Part model, mm, in its own coordinate system. A direction names the side the tool comes from. Give positions to 0.01 mm unless a question says otherwise; leave off trailing zeros. Order: outer loops, then holes, each group sorted by start corner. A loop starts at its lowest first (then second) coordinate and runs counter-clockwise, first axis right, second up. Notation, with made-up numbers: M 67.5,41 L 110.5,41 A15 ccw 110.5,67 Z; hole C 20,2.5 d10. An arc over 180 degrees is marked long. Answer as a JSON object with one key per item and string values.
from build123d import *

# Parameters (mm, degrees)
BASE_PLATE_SKETCH_W      = 35
BASE_PLATE_SKETCH_H      = 30
BASE_PLATE_DEPTH         = 10
UPRIGHT_WALL_SKETCH_W    = 35
UPRIGHT_WALL_SKETCH_H    = 7
UPRIGHT_WALL_DEPTH       = 65
TOP_PAD_SKETCH_W         = 35
TOP_PAD_SKETCH_H         = 20
TOP_PAD_DEPTH            = 6
WALL_MOUNTING_SLOT_DEPTH = 13
BEARING_BOSS_SKETCH_R    = 8
BEARING_BOSS_DEPTH       = 8
BASE_HOLE_A_SKETCH_R     = 5
BASE_HOLE_A_DEPTH        = 10
BASE_HOLE_B_SKETCH_R     = 5
BASE_HOLE_B_DEPTH        = 10
BEARING_START            = -10
BEARING_BORE_SKETCH_R    = 8
BEARING_BORE_DEPTH       = 10
WALL_TOP_FILLET_R5_A_R   = 5
WALL_TOP_FILLET_R5_B_R   = 5


with BuildPart() as part:
    # Base Plate Sketch → Base Plate (new body)
    with BuildSketch(Plane(origin=(0, 0, 0), x_dir=(1, 0, 0), z_dir=(0, 1, 0))):
        Rectangle(BASE_PLATE_SKETCH_W, BASE_PLATE_SKETCH_H)
    extrude(amount=BASE_PLATE_DEPTH)

    # Upright Wall Sketch → Upright Wall (add)
    with BuildSketch(Plane(origin=(0, 10, 0), x_dir=(1, 0, 0), z_dir=(0, 1, 0))):
        with Locations((0, 11.5)):
            Rectangle(UPRIGHT_WALL_SKETCH_W, UPRIGHT_WALL_SKETCH_H)
    extrude(amount=UPRIGHT_WALL_DEPTH)

    # Top Pad Sketch → Top Pad (add)
    with BuildSketch(Plane.XY.offset(-8)):
        with Locations((0, 65)):
            Rectangle(TOP_PAD_SKETCH_W, TOP_PAD_SKETCH_H)
    extrude(amount=TOP_PAD_DEPTH)

    # Wall Mounting Slot Sketch → Wall Mounting Slot (cut)
    with BuildSketch(Plane.XY.offset(-2)):
        with BuildLine():
            Line((-5.5, 71.124987094), (5.5, 71.124987094))
            ThreePointArc((5.5, 71.124987094), (10.5, 66.124987094), (5.5, 61.124987094))
            Line((5.5, 61.124987094), (-5.5, 61.124987094))
            ThreePointArc((-5.5, 61.124987094), (-10.5, 66.124987094), (-5.5, 71.124987094))
        make_face()
    extrude(amount=-WALL_MOUNTING_SLOT_DEPTH, mode=Mode.SUBTRACT)

    # Bearing Boss Sketch → Bearing Boss (add)
    with BuildSketch(Plane.XY.offset(-8)):
        with BuildLine():
            Line((-3, 16.837553419), (-3, 10))
            Line((-3, 10), (3, 10))
            Line((3, 10), (3, 16.837553419))
            ThreePointArc((3, 16.837553419), (0, 43.5), (-3, 16.837553419))
        make_face()
        with Locations((0, 30)):
            Circle(BEARING_BOSS_SKETCH_R, mode=Mode.SUBTRACT)
    extrude(amount=BEARING_BOSS_DEPTH)

    # Base Hole A Sketch → Base Hole A (cut)
    with BuildSketch(Plane(origin=(0, 10, 0), x_dir=(1, 0, 0), z_dir=(0, 1, 0))):
        with Locations(Location((-10.5, -7, 0), (0, 0, 270))):
            Circle(BASE_HOLE_A_SKETCH_R)
    extrude(amount=-BASE_HOLE_A_DEPTH, mode=Mode.SUBTRACT)

    # Base Hole B Sketch → Base Hole B (cut)
    with BuildSketch(Plane(origin=(0, 10, 0), x_dir=(1, 0, 0), z_dir=(0, 1, 0))):
        with Locations(Location((10.5, -7, 0), (0, 0, 270))):
            Circle(BASE_HOLE_B_SKETCH_R)
    extrude(amount=-BASE_HOLE_B_DEPTH, mode=Mode.SUBTRACT)

    # Bearing Bore Sketch → Bearing Bore (cut)
    with BuildSketch(Plane.XY.offset(-8).offset(BEARING_START)):
        with Locations((0, 30)):
            Circle(BEARING_BORE_SKETCH_R)
    extrude(amount=BEARING_BORE_DEPTH, mode=Mode.SUBTRACT)

    # Wall Top Fillet R5 A
    wall_top_fillet_r5_a_edges = [part.edges().sort_by_distance(p)[0] for p in [
        (-17.5, 75, -8.5),
    ]]
    fillet(wall_top_fillet_r5_a_edges, radius=WALL_TOP_FILLET_R5_A_R)

    # Wall Top Fillet R5 B
    wall_top_fillet_r5_b_edges = [part.edges().sort_by_distance(p)[0] for p in [
        (17.5, 75, -8.5),
    ]]
    fillet(wall_top_fillet_r5_b_edges, radius=WALL_TOP_FILLET_R5_B_R)


solid = part.part
1. Probe line 1 along Y through (x, z) = (0, -4); line 2 along X through (y, z) = (4.5, 7); line 3 along Y through (x, z) = (0, -10.5). List the from-to ranges inside material, lowest first.
Worked answers:
{"line 1": "y = 0 to 22, 38 to 43.5, 55 to 61.12, 71.12 to 75", "line 2": "x = -17.5 to -15.5, -5.5 to 5.5, 15.5 to 17.5", "line 3": "y = 0 to 22, 38 to 61.12, 71.12 to 75"}
2. Two-plate mould, pull along Y, no slides. Class faces 6 (the cylindrical face through (-16.07, 73.5, -8.59)), 7 (the cylindrical face through (-9, 5.07, 11.77)), 8 (the cylindrical face through (10.5, 66.2, -8.4)): +Y half, -Y half, draft (parallel to the pull), parting line (faces both ways), or undercut.
Worked answers:
{"face 6": "+Y half", "face 7": "draft", "face 8": "undercut"}
3. Pin check, flat tips, straight feed: P1, Ø1.5, axis at x = 7.5, z = 5, coming from the -Y side; P2, Ø6, axis at x = 1, y = 62, coming from the +Z side; P3, Ø1.5, axis at x = -5, z = 3, coming from the +Y side; P4, Ø5.5, axis at y = 13.5, z = -3.5, coming from the -X side. Stop position of each tip, or through.
Worked answers:
{"P1": "passes through", "P2": "stops at z = -2", "P3": "stops at y = 10", "P4": "stops at x = -3"}
4. Cut at C-C on z = -7. Give the cut face in (x, y), plus the area to 3 significant figures.
Worked answers:
{"outline": "M -17.5,0 L 17.5,0 L 17.5,10 L 3,10 L 3,16.84 A13.5 ccw long -3,16.84 L -3,10 L -17.5,10 Z; M -17.5,55 L 17.5,55 L 17.5,70 A5 ccw 12.5,75 L -12.5,75 A5 ccw -17.5,70 Z; hole C 0,30 d16; hole M -5.5,61.12 L 5.5,61.12 A5 ccw 5.5,71.12 L -5.5,71.12 A5 ccw Z", "area": "1,260 mm^2"}
5. Which spindle directions (+Z, -Z, +X, -X, +Y, -Y) get a long thin tool onto all of the face, cutting with end or side? Do faces 1 (the flat face through (3, 13, -4)), 2 (the flat face through (0, 55, -5)), 3 (the flat face through (0, 10, 3)), 4 (the flat face through (0, 61.125, -8)), 5 (the flat face through (6, 23, 0)). Say none if no direction does.
Worked answers:
{"face 1": "+Z, +X", "face 2": "+Z, +X, -X", "face 3": "+Z", "face 4": "+Z, -Z", "face 5": "+Z, +X, -X, +Y"}
6. Cut at A-A on z = 7. Give the cut face in (x, y), plus the area to 3 significant figures.
Worked answers:
{"outline": "M -17.5,0 L -15.5,0 L -15.5,10 L -17.5,10 Z; M -5.5,0 L 5.5,0 L 5.5,10 L -5.5,10 Z; M 15.5,0 L 17.5,0 L 17.5,10 L 15.5,10 Z", "area": "150 mm^2"}
7. Cut at D-D on y = 11. Give the cut face in (x, z), plus the area to 3 significant figures.
Worked answers:
{"outline": "M -17.5,-15 L 17.5,-15 L 17.5,-8 L 3,-8 L 3,0 L -3,0 L -3,-8 L -17.5,-8 Z", "area": "293 mm^2"}
8. Cut at B-B on y = 30. Give the cut face in (x, z), plus the area to 3 significant figures.
Worked answers:
{"outline": "M -17.5,-15 L -8,-15 L -8,0 L -13.5,0 L -13.5,-8 L -17.5,-8 Z; M 8,-15 L 17.5,-15 L 17.5,-8 L 13.5,-8 L 13.5,0 L 8,0 Z", "area": "221 mm^2"}
